Source: three-view drawing plus pictorial views. Frame: mm from the lowest corner of the part. A direction names the side the tool comes from. Give positions to 0.01 mm unless a question says otherwise; leave off trailing zeros. Loops run counter-clockwise (first coordinate to the right, second up) from the corner with the lowest first, then second, coordinate; pieces in that order, holes last. Notation, with made-up numbers: (48, -18.75) - (89, -18.75) arc R26 ccw to (89, -3.75) - close; hole circle Ø9 at (49, 9.5). An arc over 180 degrees is marked (long way). Answer as a JSON object with one key per item and string values. Group by question number.
(1) Section query D-D (y = 23.5). Return loops of the section in (x, z) (1 decimal).
(2) Section query B-B (z = 27.5). Return loops of the section in (x, y) (1 decimal).
(3) Pin query (flat end, axial travel): P1, Ø12, axis at x = 32, y = 28.5, coming from the -Z side; P2, Ø1.5, axis at y = 39, z = 18, coming from the -X side; P3, Ø20.5, axis at x = 44, y = 29, coming from the +Z side; P4, Ø1, axis at y = 31, z = 22, coming from the -X side. Return the tip coordinate at first contact, or that it passes through.
(4) Section query C-C (x = 108). Return loops of the section in (y, z), plus the area to 3 significant figures.
(5) Access query for the marked faces 1, 2, 3 and 4. Directions: +Z, -Z, +X, -X, +Y, -Y. A direction counts if a zero-diameter tool reaches every point of the face in a straight line with its end or side. Return the directions, or none.
(6) Section query A-A (y = 31.5). Return loops of the section in (x, z) (1 decimal).
(7) Material intervals for L1, parallel to Z at x = 21, y = 25; L2, parallel to Z at x = 31, y = 2.5; L3, parallel to Y at x = 11, z = 9, sorted ascending.
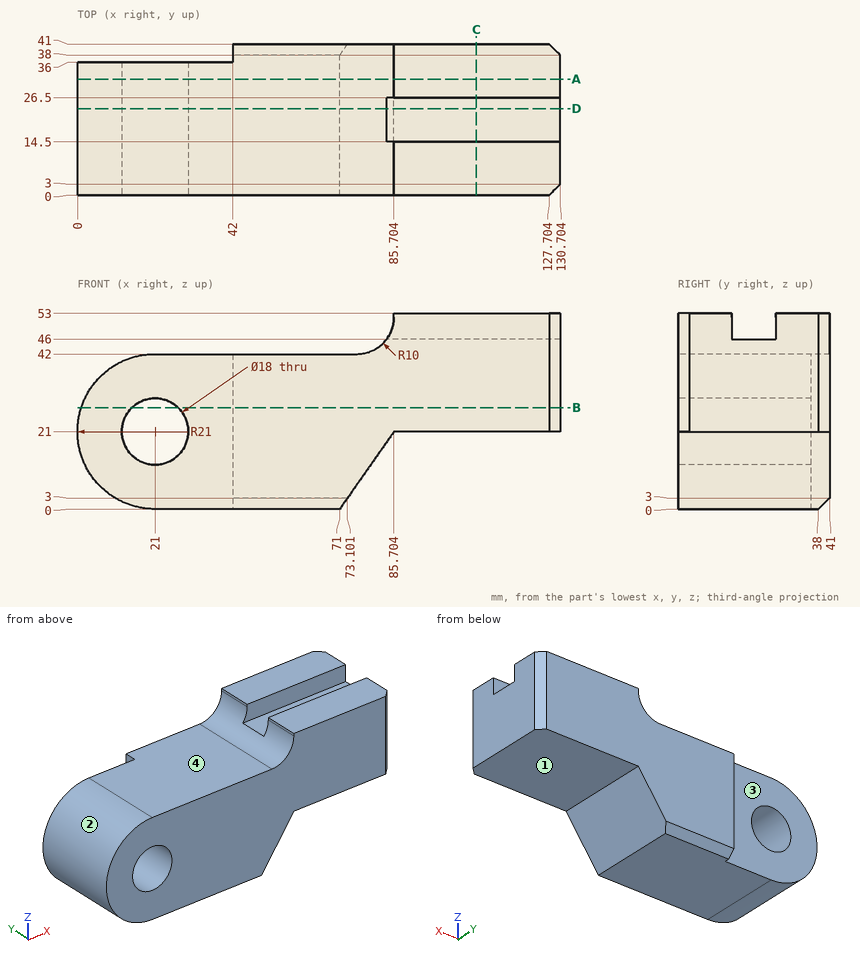
Recorded:
{
 "1": {"outline": "(21, 0) - (71, 0) - (85.7, 21) - (130.7, 21) - (130.7, 46) - (83.7, 46) arc R10 cw to (75.7, 42) - (21, 42) arc R21 ccw to start; hole circle Ø18 at (21, 21)"},
 "2": {"outline": "(1, 0) - (14.8, 0) - (14.8, 36) - (1, 36) - close; (27.2, 0) - (127.7, 0) - (130.7, 3) - (130.7, 38) - (127.7, 41) - (42, 41) - (42, 36) - (27.2, 36) - close"},
 "3": {"P1": "stops at z = 0", "P2": "stops at x = 42", "P3": "stops at z = 42", "P4": "stops at x = 0.01"},
 "4": {"outline": "(0, 21) - (41, 21) - (41, 53) - (26.5, 53) - (26.5, 46) - (14.5, 46) - (14.5, 53) - (0, 53) - close", "area": "1,230 mm^2"},
 "5": {"face 1": "-Z, +X, +Y, -Y", "face 2": "-X, +Y, -Y", "face 3": "+Z, -Z, -X, +Y", "face 4": "+Z, -X, +Y, -Y"},
 "6": {"outline": "(21, 0) - (71, 0) - (85.7, 21) - (130.7, 21) - (130.7, 53) - (85.7, 53) - (85.7, 52) arc R10 cw to (75.7, 42) - (21, 42) arc R21 ccw to start; hole circle Ø18 at (21, 21)"},
 "7": {"L1": "z = 0 to 12, 30 to 42", "L2": "z = 0 to 42", "L3": "y = 0 to 36"}
}
